Part model, mm, in its own coordinate system. Round coordinates to 2 decimals unless told otherwise and drop trailing zeros. Loops run counter-clockwise (first coordinate to the right, second up) from the corner with the lowest first, then second, coordinate; pieces in that order, holes last. Notation, with made-up numbers: (42.5, 18.25) -> (61.5, 18.25) arc R36 ccw to (61.5, 52.25) -> close; hole circle Ø3 at (26.25, 44). An arc over 180 degrees is marked (long way). Answer as CSV lines item,"result".
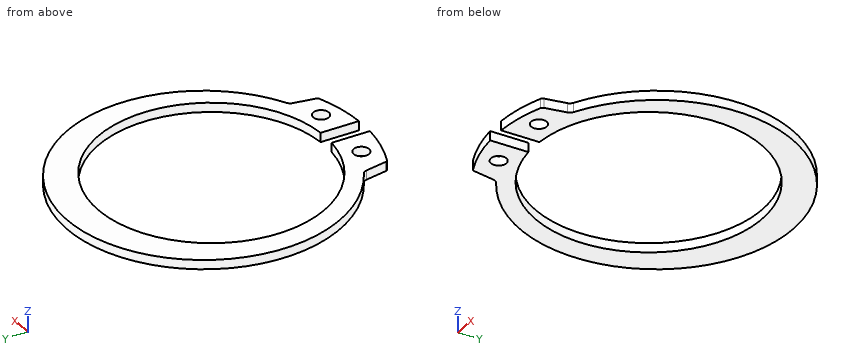
from build123d import *

# Parameters (mm, degrees)
EXTRUDE_972_DEPTH      = 0.75
EXTRUDE_972_DEPTH_BACK = 0.75
SKETCH_1_R             = 1.25


with BuildPart() as part:
    # 草图1 → Extrude 972 (new, two sides: drawn at the far end of the back side and taken through both)
    with BuildSketch(Plane.XY.offset(-EXTRUDE_972_DEPTH_BACK)):
        with BuildLine():
            Line((-1.5, -19.438251703), (-1.5, -25.503659518))
            ThreePointArc((-1.5, -25.503659518), (-5.420429348, -24.937738298), (-9.196831336, -23.742405238))
            ThreePointArc((-9.196831336, -23.742405238), (-9.396824452, -23.593447727), (-9.5, -23.366422634))
            Line((-9.5, -23.366422634), (-10.097014043, -19.980587746))
            ThreePointArc((-10.097014043, -19.980587746), (-10.268699557, -19.572142955), (-10.600003457, -19.277964797))
            ThreePointArc((-10.600003457, -19.277964797), (0, 22), (10.600003457, -19.277964797))
            ThreePointArc((10.600003457, -19.277964797), (10.268699557, -19.572142955), (10.097014043, -19.980587746))
            Line((10.097014043, -19.980587746), (9.5, -23.366422634))
            ThreePointArc((9.5, -23.366422634), (9.396824452, -23.593447727), (9.196831336, -23.742405238))
            ThreePointArc((9.196831336, -23.742405238), (5.420429348, -24.937738298), (1.5, -25.503659518))
            Line((1.5, -25.503659518), (1.5, -19.438251703))
            ThreePointArc((1.5, -19.438251703), (0, 17), (-1.5, -19.438251703))
        make_face()
        with Locations((-5.5, -21.827657787)):
            Circle(SKETCH_1_R, mode=Mode.SUBTRACT)
        with Locations(Location((5.5, -21.827657787, 0), (0, 0, 180))):
            Circle(SKETCH_1_R, mode=Mode.SUBTRACT)
    extrude(amount=EXTRUDE_972_DEPTH + EXTRUDE_972_DEPTH_BACK)


solid = part.part
Q1. Saw through at C-C, the plane z = 0.1. Write the cut outline in (x, y).
Geometry results:
outline,"(-10.6, -19.28) arc R1 cw to (-10.1, -19.98) -> (-9.5, -23.37) arc R0.5 ccw to (-9.2, -23.74) arc R24.3 ccw to (-1.5, -25.5) -> (-1.5, -19.44) arc R18.25 cw (long way) to (1.5, -19.44) -> (1.5, -25.5) arc R24.3 ccw to (9.2, -23.74) arc R0.5 ccw to (9.5, -23.37) -> (10.1, -19.98) arc R1 cw to (10.6, -19.28) arc R22 ccw (long way) to start; hole circle Ø2.5 at (-5.5, -21.83); hole circle Ø2.5 at (5.5, -21.83)"
Q2. Saw through at B-B, the plane x = -5.5. Write the cut outline in (y, z).
Geometry results:
outline,"(-24.92, -0.75) -> (-23.08, -0.75) -> (-23.08, 0.75) -> (-24.92, 0.75) -> close; (-20.58, -0.75) -> (-18.65, -0.75) -> (-18.65, 0.75) -> (-20.58, 0.75) -> close; (16.15, -0.75) -> (21.3, -0.75) -> (21.3, 0.75) -> (16.15, 0.75) -> close"
Q3. Drill centre lines: line 1 along Y through (x, z) = (-5.5, 0.2); line 2 along Y through (x, z) = (5, 0.55); line 3 along X through (y, z) = (15, -0.6). Where is each one in solid material? Low to high.
Geometry results:
line 1,"-24.92 to -23.08, -20.58 to -18.65, 16.15 to 21.3"
line 2,"-25.03 to -22.97, -20.68 to -18.8, 16.3 to 21.42"
line 3,"-16.09 to -8.31, 8.31 to 16.09"
Q4. Saw through at D-D, the plane y = -1.25. Write the cut outline in (x, z).
Geometry results:
outline,"(-21.96, -0.75) -> (-18.25, -0.75) -> (-18.25, 0.75) -> (-21.96, 0.75) -> close; (18.25, -0.75) -> (21.96, -0.75) -> (21.96, 0.75) -> (18.25, 0.75) -> close"
Q5. Saw through at A-A, the plane y = 5. Write the cut outline in (x, z).
Geometry results:
outline,"(-21.42, -0.75) -> (-17.15, -0.75) -> (-17.15, 0.75) -> (-21.42, 0.75) -> close; (17.15, -0.75) -> (21.42, -0.75) -> (21.42, 0.75) -> (17.15, 0.75) -> close"
